Can you work these out from the model? Positions are in its coordinate system, mm. A direction names the side the tool comes from. Round coordinates to 2 decimals unless told otherwise and drop trailing zeros. Loops run counter-clockwise (first coordinate to the right, second up) from the corner with the lowest first, then second, coordinate; pieces in that order, holes last. Notation, with made-up numbers: (4.5, 53.5) -> (32.5, 53.5) arc R17 ccw to (32.5, 84.5) -> close; hole circle Ø7 at (-25.5, 69.5). An arc over 180 degrees is marked (long way). Use a Markdown table: item, result.
from build123d import *

# Parameters (mm, degrees)
FORK_BODY_PROFILE_SKETCH_R      = 9
FORK_BODY_DEPTH                 = 44
OFFSET_TANG_SKETCH_W            = 50
OFFSET_TANG_SKETCH_H            = 54
OFFSET_TANG_DEPTH               = 15
TANG_CROSS_HOLE_REACH           = 128.574
TANG_CROSS_HOLE_SKETCH_R        = 10
TANG_SLOT_2MM_REACH             = 138.429
TANG_SLOT_SKETCH_W              = 34
TANG_SLOT_SKETCH_H              = 2
FORK_ROOT_FILLET_R14_R          = 14
SIDE_RELIEF_SKETCH_R            = 3.5
SIDE_RELIEF_CUT_DEPTH           = 50
FORK_EYE_PROFILE_CUT_DEPTH      = 127.574088976
FORK_EYE_PROFILE_CUT_DEPTH_BACK = 127.574088976


with BuildPart() as part:
    # Fork Body Profile Sketch → Fork Body (new, symmetric)
    with BuildSketch(Plane(origin=(0, 0, 0), x_dir=(1, 0, 0), z_dir=(0, 1, 0))):
        with BuildLine():
            Line((0, -24), (-64, -24))
            Line((-64, -24), (-64, -9))
            Line((-64, -9), (-35.874782229, -9))
            ThreePointArc((-35.874782229, -9), (-27.750743825, -5.831760866), (-23.916521486, 2))
            ThreePointArc((-23.916521486, 2), (17.663521733, 16.248076809), (0, -24))
        make_face()
        with Locations(Location((0, 0, 0), (0, 0, 270))):
            Circle(FORK_BODY_PROFILE_SKETCH_R, mode=Mode.SUBTRACT)
    extrude(amount=FORK_BODY_DEPTH, both=True)

    # Offset Tang Sketch → Offset Tang (add)
    with BuildSketch(Plane(origin=(0, 0, 9), x_dir=(-1, 0, 0), z_dir=(0, 0, -1))):
        with Locations((89, 0)):
            Rectangle(OFFSET_TANG_SKETCH_W, OFFSET_TANG_SKETCH_H)
    extrude(amount=-OFFSET_TANG_DEPTH)

    # Tang Cross Hole Sketch → Tang Cross Hole (cut, up to next)
    with BuildSketch(Plane(origin=(0, 0, 9), x_dir=(-1, 0, 0), z_dir=(0, 0, -1)), mode=Mode.PRIVATE) as tang_cross_hole_sk1:
        with Locations((97, 0)):
            Circle(TANG_CROSS_HOLE_SKETCH_R)
    tang_cross_hole_tool1 = extrude(tang_cross_hole_sk1.sketch, amount=-TANG_CROSS_HOLE_REACH, mode=Mode.PRIVATE) & part.part
    add(tang_cross_hole_tool1.solids().sort_by_distance((-97, 0, 9))[0], mode=Mode.SUBTRACT)

    # Tang Slot Sketch → Tang Slot 2mm (cut, up to next)
    with BuildSketch(Plane.XZ.offset(27), mode=Mode.PRIVATE) as tang_slot_2mm_sk1:
        with Locations((-97, 16.5)):
            Rectangle(TANG_SLOT_SKETCH_W, TANG_SLOT_SKETCH_H)
    tang_slot_2mm_tool1 = extrude(tang_slot_2mm_sk1.sketch, amount=-TANG_SLOT_2MM_REACH, mode=Mode.PRIVATE) & part.part
    add(tang_slot_2mm_tool1.solids().sort_by_distance((-97, -27, 16.5))[0], mode=Mode.SUBTRACT)

    # Fork Root Fillet R14
    fork_root_fillet_r14_edges = [part.edges().sort_by_distance(p)[0] for p in [
        (-64, -27, 16.5),
        (-64, 27, 16.5),
    ]]
    fillet(fork_root_fillet_r14_edges, radius=FORK_ROOT_FILLET_R14_R)

    # Side Relief Sketch → Side Relief Cut (cut)
    with BuildSketch(Plane.ZY.offset(114)):
        with Locations((16.5, 17)):
            Circle(SIDE_RELIEF_SKETCH_R)
        with Locations(Location((16.5, -17, 0), (0, 0, 73.398450401))):
            Circle(SIDE_RELIEF_SKETCH_R)
    extrude(amount=-SIDE_RELIEF_CUT_DEPTH, mode=Mode.SUBTRACT)

    # Fork Eye Profile Sketch → Fork Eye Profile Cut (cut, two sides: drawn at the far end of the back side and taken through both)
    with BuildSketch(Plane(origin=(0, 0, 9), x_dir=(-1, 0, 0), z_dir=(0, 0, -1)).offset(-FORK_EYE_PROFILE_CUT_DEPTH_BACK)):
        with BuildLine():
            Line((-24, 22), (52, 22))
            ThreePointArc((52, 22), (60.485281374, 18.485281374), (64, 10))
            Line((64, 10), (64, -10))
            ThreePointArc((64, -10), (60.485281374, -18.485281374), (52, -22))
            Line((52, -22), (-24, -22))
            Line((-24, -22), (-24, 22))
        make_face()
    extrude(amount=FORK_EYE_PROFILE_CUT_DEPTH + FORK_EYE_PROFILE_CUT_DEPTH_BACK, mode=Mode.SUBTRACT)


solid = part.part
1. If we mould it in two halves opening along Y, with no side actions, what happens to faces 1 (the cylindrical face through (-27.843, -32.846, 5.916)), 2 (the flat face through (-10, -44, 5)), 3 (the cylindrical face through (-60.39, 18.58, 16.61))? For each: +Y half, -Y half, draft (parallel to the pull), parting line (faces both ways), or undercut.
Answer sheet:
| item | result |
|---|---|
| face 1 | draft |
| face 2 | -Y half |
| face 3 | undercut |
2. I need wall thicknesses on line 1 (Y direction, x = -77.5, z = 16.5); line 2 (Y direction, x = -0.5, z = 17); line 3 (Z direction, x = -81.5, y = 4). Which ranges of each line are inside material? Lowest first, please.
Answer sheet:
| item | result |
|---|---|
| line 1 | y = -27.01 to -20.5, -13.5 to 13.5, 20.5 to 27.01 |
| line 2 | y = -44 to -22, 22 to 44 |
| line 3 | z = 9 to 15.5, 17.5 to 24 |
3. Will these pins go through, and if not, where does the flat tip stop? pin 1 Ø7.5 at (x, y) = (-98, 25) entering from -Z; pin 2 Ø3 at (x, z) = (-85, 15) entering from +Y; pin 3 Ø2.5 at (y, z) = (-42, 13) entering from -X.
Answer sheet:
| item | result |
|---|---|
| pin 1 | stops at z = 9 |
| pin 2 | stops at y = 27 |
| pin 3 | stops at x = -64 |
4. I want a section at C-C (z = 4.5). Please give me the cut outline in (x, y), plus the area to 3 significant figures.
Answer sheet:
| item | result |
|---|---|
| outline | (-26.51, -44) -> (-7.79, -44) -> (-7.79, -22) -> (-26.51, -22) -> close; (-26.51, 22) -> (-7.79, 22) -> (-7.79, 44) -> (-26.51, 44) -> close; (7.79, -44) -> (23.57, -44) -> (23.57, -22) -> (7.79, -22) -> close; (7.79, 22) -> (23.57, 22) -> (23.57, 44) -> (7.79, 44) -> close |
| area | 1,520 mm² |
5. I want a section at A-A (y = 0). Please give me the cut outline in (x, z), plus the area to 3 significant figures.
Answer sheet:
| item | result |
|---|---|
| outline | (-114, 9) -> (-107, 9) -> (-107, 15.5) -> (-114, 15.5) -> close; (-114, 17.5) -> (-107, 17.5) -> (-107, 24) -> (-114, 24) -> close; (-87, 9) -> (-64, 9) -> (-64, 24) -> (-87, 24) -> (-87, 17.5) -> (-80, 17.5) -> (-80, 15.5) -> (-87, 15.5) -> close |
| area | 422 mm² |
6. Which directions (+Z, -Z, +X, -X, +Y, -Y) give clear straight access to the entire face, cutting with the end or side of a thin tool? Please do faces 4 (the flat face through (-97, 24, 17.5)), 5 (the flat face through (-96, -27, 15)), 6 (the cylindrical face through (-89.35, -20.307, 15.353)), 7 (the flat face through (-75, 1, 9)).
Answer sheet:
| item | result |
|---|---|
| face 4 | -X, +Y, -Y |
| face 5 | +Z, -Z, -X, -Y |
| face 6 | -X |
| face 7 | -Z, -X, +Y, -Y |
7. I want a section at D-D (z = -13). Please give me the cut outline in (x, y).
Answer sheet:
| item | result |
|---|---|
| outline | (-20.17, -44) -> (20.17, -44) -> (20.17, -22) -> (-20.17, -22) -> close; (-20.17, 22) -> (20.17, 22) -> (20.17, 44) -> (-20.17, 44) -> close |
8. I want a section at B-B (x = -89.5). Please give me the cut outline in (y, z), plus the area to 3 significant figures.
Answer sheet:
| item | result |
|---|---|
| outline | (-27, 9) -> (-6.61, 9) -> (-6.61, 15.5) -> (-13.65, 15.5) arc R3.5 cw to (-20.35, 15.5) -> (-27, 15.5) -> close; (-27, 17.5) -> (-20.35, 17.5) arc R3.5 cw to (-13.65, 17.5) -> (-6.61, 17.5) -> (-6.61, 24) -> (-27, 24) -> close; (6.61, 9) -> (27, 9) -> (27, 15.5) -> (20.35, 15.5) arc R3.5 cw to (13.65, 15.5) -> (6.61, 15.5) -> close; (6.61, 17.5) -> (13.65, 17.5) arc R3.5 cw to (20.35, 17.5) -> (27, 17.5) -> (27, 24) -> (6.61, 24) -> close |
| area | 481 mm² |
